from build123d import *

# Parameters (mm, degrees)
HEX_BODY_3MM_DEPTH      = 3
BORE_PROFILE_8_R        = 4
BORE_8_DEPTH            = 3
HEX_CORNER_FILLETS_R1_R = 1


with BuildPart() as part:
    # Hex Profile 14AF → Hex Body 3mm (new body)
    with BuildSketch(Plane(origin=(0, 0, 0), x_dir=(1, 0, 0), z_dir=(0, 1, 0))):
        Polygon((0, 8.082903769), (-7, 4.041451884), (-7, -4.041451884), (0, -8.082903769), (7, -4.041451884), (7, 4.041451884), align=None)
    extrude(amount=HEX_BODY_3MM_DEPTH)

    # Bore Profile Ø8 → Bore Ø8 (cut)
    with BuildSketch(Plane(origin=(0, 3, 0), x_dir=(1, 0, 0), z_dir=(0, 1, 0))):
        with Locations(Location((0, 0, 0), (0, 0, 270))):
            Circle(BORE_PROFILE_8_R)
    extrude(amount=-BORE_8_DEPTH, mode=Mode.SUBTRACT)

    # Hex Corner Fillets R1
    hex_corner_fillets_r1_edges = [part.edges().sort_by_distance(p)[0] for p in [
        (7, 1.5, -4.041451884),
        (7, 1.5, 4.041451884),
        (0, 1.5, 8.082903769),
        (-7, 1.5, 4.041451884),
        (-7, 1.5, -4.041451884),
        (0, 1.5, -8.082903769),
    ]]
    fillet(hex_corner_fillets_r1_edges, radius=HEX_CORNER_FILLETS_R1_R)


solid = part.part
Work out the finished part from the listing and answer in its coordinate system (mm). Coordinates: 2 decimals unless noted, no trailing zeros. Loops run counter-clockwise (first coordinate to the right, second up) from the corner with the lowest first, then second, coordinate; pieces in that order, holes last. Notation, with made-up numbers: (50.5, 11.5) -> (65.5, 11.5) arc R13 ccw to (65.5, 25.5) -> close; hole circle Ø4 at (-4.75, -38). An arc over 180 degrees is marked (long way). Write each question's results on one line, items separated by ' | '. Start each with the question number.
1) Consider line 1 along X through (y, z) = (0.75, 0); line 2 along X through (y, z) = (1.4, 3); line 3 along Z through (x, y) = (-1.5, 2.2). Determine where each line is inside the solid, lowest interval first.
2) Find section B-B on x = 0. Determine the outline of the cut face in (y, z), then the cut area to 3 significant figures.
3) A flat-ended cylindrical pin translates along its axis: P1, Ø1.5, axis at x = -2, y = 2.5, coming from the +Z side. Find the tip coordinate at first contact, or state that the pin passes through.
4) Find section C-C on z = 0. Determine the outline of the cut face in (x, y).
5) The mould has two halves that part along Z. Classify faces 1 (the flat face through (-3.54, 1.48, 6.04)), 2 (the flat face through (-3.458, 1.479, -6.086)), 3 (the flat face through (3, 3, 3)), 4 (the cylindrical face through (-3.905, 1.521, -0.867)): pulls with the +Z half, pulls with the -Z half, needs draft (parallel to the pull), parting line crosses it, or undercut.
6) Find section D-D on z = 6.75. Determine the outline of the cut face in (x, y), then the cut area to 3 significant figures.
7) Find section A-A on y = 2.05. Determine the outline of the cut face in (x, z).
Response values:
1) line 1: x = -7 to -4, 4 to 7 | line 2: x = -7 to -2.65, 2.65 to 7 | line 3: z = -7.22 to -3.71, 3.71 to 7.22
2) outline: (0, -7.93) -> (3, -7.93) -> (3, -4) -> (0, -4) -> close; (0, 4) -> (3, 4) -> (3, 7.93) -> (0, 7.93) -> close | area: 23.6 mm^2
3) P1: stops at z = 7.36
4) outline: (-7, 0) -> (-4, 0) -> (-4, 3) -> (-7, 3) -> close; (4, 0) -> (7, 0) -> (7, 3) -> (4, 3) -> close
5) face 1: pulls with the +Z half | face 2: pulls with the -Z half | face 3: needs draft | face 4: undercut
6) outline: (-2.31, 0) -> (2.31, 0) -> (2.31, 3) -> (-2.31, 3) -> close | area: 13.9 mm^2
7) outline: (-7, -3.46) arc R1 ccw to (-6.5, -4.33) -> (-0.5, -7.79) arc R1 ccw to (0.5, -7.79) -> (6.5, -4.33) arc R1 ccw to (7, -3.46) -> (7, 3.46) arc R1 ccw to (6.5, 4.33) -> (0.5, 7.79) arc R1 ccw to (-0.5, 7.79) -> (-6.5, 4.33) arc R1 ccw to (-7, 3.46) -> close; hole circle Ø8 at (0, 0)
